from build123d import *

# Parameters (mm, degrees)
BASE_DISC_SKETCH_R                          = 38
BASE_DISC_76X18_DEPTH                       = 9
SPIGOT_SKETCH_R                             = 24
SPIGOT_48X8_DEPTH                           = 4
COUNTERBORED_MOUNTING_HOLES_5_3_D           = 5.3
COUNTERBORED_MOUNTING_HOLES_5_3_CBORE_D     = 7.8
COUNTERBORED_MOUNTING_HOLES_5_3_CBORE_DEPTH = 4
COUNTERBORE_BORE_SKETCH_R                   = 19
COUNTERBORE_BORE_38X16_DEPTH                = 8
THROUGH_BORE_28_REACH                       = 57.534
THROUGH_BORE_SKETCH_R                       = 14
BORE_EDGE_FILLET_R2_R                       = 2
RADIAL_HOLE_5X20_D                          = 5
RADIAL_HOLE_5X20_DEPTH                      = 20


with BuildPart() as part:
    # Base Disc Sketch → Base Disc Ø76x18 (new, symmetric)
    with BuildSketch(Plane(origin=(0, 0, 0), x_dir=(1, 0, 0), z_dir=(0, 1, 0))):
        with Locations(Location((0, 0, 0), (0, 0, 270))):
            Circle(BASE_DISC_SKETCH_R)
    extrude(amount=BASE_DISC_76X18_DEPTH, both=True)

    # Spigot Sketch → Spigot Ø48x8 (add, symmetric)
    with BuildSketch(Plane(origin=(0, 9, 0), x_dir=(1, 0, 0), z_dir=(0, 1, 0))):
        with Locations(Location((0, 0, 0), (0, 0, 270))):
            Circle(SPIGOT_SKETCH_R)
    extrude(amount=SPIGOT_48X8_DEPTH, both=True)

    # Counterbored Mounting Holes Ø5.3 (through all)
    with Locations(Plane(origin=(0, -9, 28), x_dir=(0, 0, -1), z_dir=(0, -1, 0))):
        with Locations((0, 0), (28, 28), (56, 0), (28, -28)):
            CounterBoreHole(COUNTERBORED_MOUNTING_HOLES_5_3_D / 2, COUNTERBORED_MOUNTING_HOLES_5_3_CBORE_D / 2, COUNTERBORED_MOUNTING_HOLES_5_3_CBORE_DEPTH)

    # Counterbore Bore Sketch → Counterbore Bore Ø38x16 (cut, symmetric)
    with BuildSketch(Plane.XZ.offset(9)):
        with Locations(Location((0, 0, 0), (0, 0, 270))):
            Circle(COUNTERBORE_BORE_SKETCH_R)
    extrude(amount=COUNTERBORE_BORE_38X16_DEPTH, both=True, mode=Mode.SUBTRACT)

    # Through Bore Sketch → Through Bore Ø28 (cut, up to next)
    with BuildSketch(Plane.XZ.offset(1), mode=Mode.PRIVATE) as through_bore_28_sk1:
        with Locations(Location((0, 0, 0), (0, 0, 270))):
            Circle(THROUGH_BORE_SKETCH_R)
    through_bore_28_tool1 = extrude(through_bore_28_sk1.sketch, amount=-THROUGH_BORE_28_REACH, mode=Mode.PRIVATE) & part.part
    add(through_bore_28_tool1.solids().sort_by_distance((0, -1, 0))[0], mode=Mode.SUBTRACT)

    # Bore Edge Fillet R2
    bore_edge_fillet_r2_edges = [part.edges().sort_by_distance(p)[0] for p in [
        (0, -1, 19),
    ]]
    fillet(bore_edge_fillet_r2_edges, radius=BORE_EDGE_FILLET_R2_R)

    # Radial Hole Ø5x20
    with Locations(Plane(origin=(19, 0, 32.908965344), x_dir=(0.8660254037844379, 0, -0.5000000000000013), z_dir=(0.5000000000000013, 0, 0.8660254037844379))):
        with Locations((0, 0)):
            Hole(RADIAL_HOLE_5X20_D / 2, depth=RADIAL_HOLE_5X20_DEPTH)


solid = part.part
CAD build for the part. Positions are in the model's coordinates, mm. A direction names the side the tool comes from. Coordinates: 2 decimals unless noted, no trailing zeros. Loops run counter-clockwise (first coordinate to the right, second up) from the corner with the lowest first, then second, coordinate; pieces in that order, holes last. Notation, with made-up numbers: (-35, 31) -> (-31, 31) arc R19 ccw to (-31, 64) -> close; hole circle Ø6 at (46.25, -19.75). An arc over 180 degrees is marked (long way). One line per item, written item: value.
1. Slice it at A-A on x = 0. Give the number of separate pieces and of enclosed holes in the cut face, and give its area (3 significant figures).
Answers:
separate pieces: 4
enclosed holes: 0
area: 655 mm^2
2. Slice it at C-C on y = 7.25. Write the cut outline in (x, z).
Answers:
outline: circle Ø76 at (0, 0); hole circle Ø5.3 at (-28, 0); hole circle Ø28 at (0, 0); hole circle Ø5.3 at (0, -28); hole circle Ø5.3 at (0, 28); hole circle Ø5.3 at (28, 0)
3. Which spindle directions (+Z, -Z, +X, -X, +Y, -Y) get a long thin tool onto all of the face, cutting with end or side? Do faces 4 (the face through (-11.56, -6.04, 15.08)), 5 (the face through (-25.37, 2.1, -0.34)). Say none if no direction does.
Answers:
face 4: -Y
face 5: +Y, -Y
4. Drill centre lines: line 1 (X direction, y = -8.05, z = 0); line 2 (X direction, y = 3.5, z = 0); line 3 (X direction, y = 4.5, z = 8). Where is each one in solid material? Low to high. Write a range as [from, to].
Answers:
line 1: x = [-38, -31.9], [-24.1, -19], [19, 24.1], [31.9, 38]
line 2: x = [-38, -30.65], [-25.35, -14], [14, 25.35], [30.65, 38]
line 3: x = [-37.15, -11.49], [11.49, 37.15]
5. Slice it at D-D on x = -28. Write the cut outline in (y, z).
Answers:
outline: (-9, -25.69) -> (9, -25.69) -> (9, -2.65) -> (-5, -2.65) -> (-5, -3.9) -> (-9, -3.9) -> close; (-9, 3.9) -> (-5, 3.9) -> (-5, 2.65) -> (9, 2.65) -> (9, 25.69) -> (-9, 25.69) -> close
6. Pull direction X, two halves, no side cores. Call faces 1 (the face through (30.63, 2.1, -0.34)), 2 (the face through (1, 9, 25)), 3 (the face through (7.21, 11.03, 22.89)): pulls with the +X half, pulls with the -X half, needs draft (parallel to the pull), parting line crosses it, or undercut.
Answers:
face 1: undercut
face 2: needs draft
face 3: parting line crosses it
7. Flat gauge pins, fed straight in: P1, Ø4, axis at x = 30, z = 0.5, coming from the -Y side; P2, Ø22.5, axis at x = 0, z = 0, coming from the +Y side; P3, Ø6, axis at x = -12, y = 10.5, coming from the +Z side; P4, Ø2, axis at y = 1, z = 18.5, coming from the -X side. Where does each tip first touch, or does it go through?
Answers:
P1: stops at y = -9
P2: passes through
P3: stops at z = 36.82
P4: stops at x = -33.73
